```python
from build123d import *

# Parameters (mm, degrees)
SKETCH1_W           = 90
SKETCH1_H           = 90
BOSS_EXTRUDE1_DEPTH = 7.5
SKETCH2_R           = 19
CUT_EXTRUDE1_DEPTH  = 15


with BuildPart() as part:
    # Sketch1 → Boss-Extrude1 (new, symmetric)
    with BuildSketch(Plane(origin=(0, 0, 0), x_dir=(0, 0, -1), z_dir=(1, 0, 0))):
        Rectangle(SKETCH1_W, SKETCH1_H)
    extrude(amount=BOSS_EXTRUDE1_DEPTH, both=True)

    # Sketch2 → Cut-Extrude1 (cut)
    with BuildSketch(Plane(origin=(7.5, 0, 0), x_dir=(0, 0, -1), z_dir=(1, 0, 0))):
        with Locations((-15, 5)):
            Circle(SKETCH2_R)
    extrude(amount=-CUT_EXTRUDE1_DEPTH, mode=Mode.SUBTRACT)


solid = part.part
```
Could you check a few things on this model? Use its own coordinates, in mm. Round coordinates to 2 decimals unless told otherwise and drop trailing zeros. Write each loop counter-clockwise with the first axis right and the second up, starting at its lowest first coordinate (ties: lowest second). Pieces come first, ordered by that corner, then holes.
(1) If I drill on probe 1 along Y at (x, z) = (-0.5, 15); probe 2 along Y at (x, z) = (1.5, 24); probe 3 along Z at (x, y) = (-0.25, -3), over which ranges is the centre line in solid material (lowest first)?
Findings below:
probe 1: y = -45 to -14, 24 to 45
probe 2: y = -45 to -11.73, 21.73 to 45
probe 3: z = -45 to -2.23, 32.23 to 45
(2) Suppose I cut it at B-B on z = 15. Write out the boundary of the cut face in (x, y), and give its area (3 significant figures).
Findings below:
outline: (-7.5, -45) - (7.5, -45) - (7.5, -14) - (-7.5, -14) - close; (-7.5, 24) - (7.5, 24) - (7.5, 45) - (-7.5, 45) - close
area: 780 mm2
(3) Suppose I cut it at A-A on y = 5. Write out the boundary of the cut face in (x, z).
Findings below:
outline: (-7.5, -45) - (7.5, -45) - (7.5, -4) - (-7.5, -4) - close; (-7.5, 34) - (7.5, 34) - (7.5, 45) - (-7.5, 45) - close
(4) Suppose I cut it at C-C on x = 5.5. Write out the boundary of the cut face in (y, z).
Findings below:
outline: (-45, -45) - (45, -45) - (45, 45) - (-45, 45) - close; hole circle Ø38 at (5, 15)
